Verification items for this drawing (mm, ordinates from the low corner). A direction names the side the tool comes from. Round coordinates to 2 decimals unless told otherwise and drop trailing zeros. Write each loop counter-clockwise with the first axis right and the second up, starting at its lowest first coordinate (ties: lowest second). Pieces come first, ordered by that corner, then holes. Notation, with made-up numbers: (15, 62) -> (30, 62) arc R20 cw to (30, 86) -> close; hole circle Ø6 at (75, -13). An arc over 180 degrees is marked (long way). One line per item, written item: value.
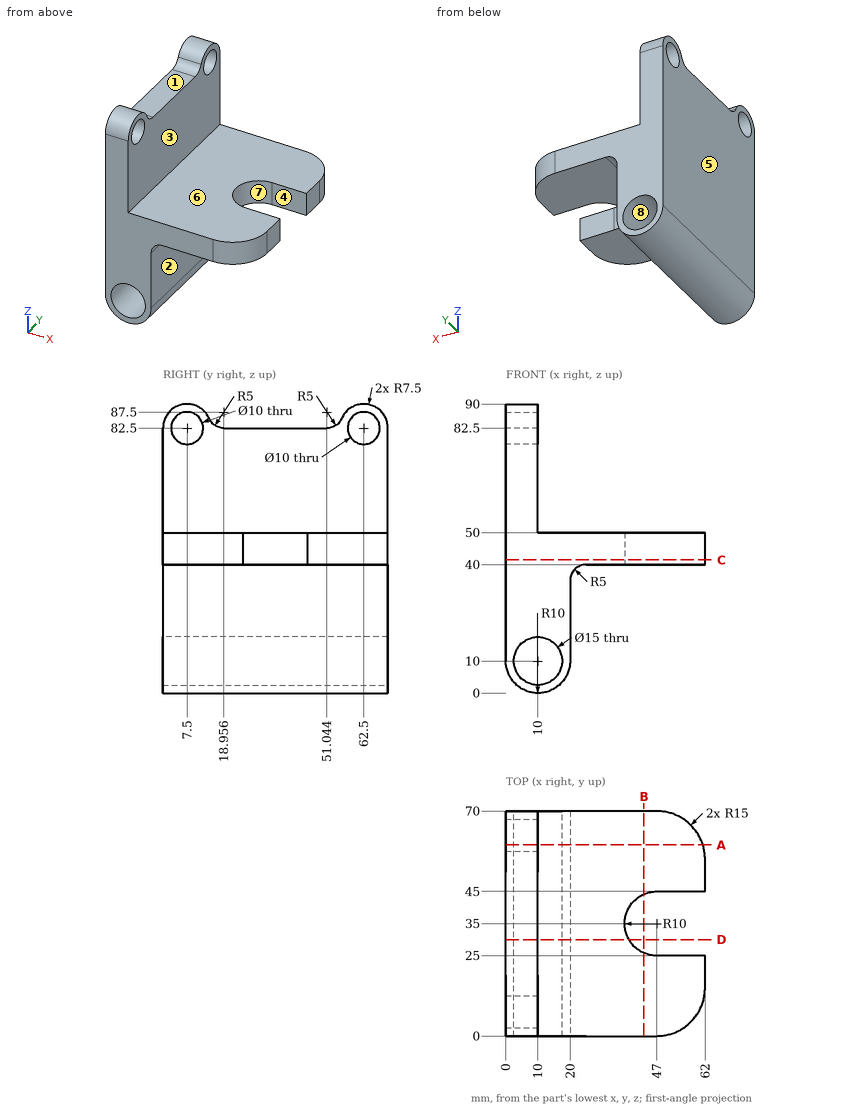
Item 1: Depth check by flat-ended pin: pin 1 (3 mm diameter, centred on x = 13.5, y = 32, fed in from +Z); pin 2 (9 mm diameter, centred on x = 10, z = 10, fed in from +Y); pin 3 (12 mm diameter, centred on x = 28.5, y = 62, fed in from -Z); pin 4 (3 mm diameter, centred on x = 58, z = 45, fed in from +Y). Enter the tip coordinate at first touch or a pass-through.
Result set:
pin 1: z = 50
pin 2: through
pin 3: z = 39.33
pin 4: y = 66.61
Item 2: Sectioned sample at A-A (y = 59.5). Enter the section's corners in (x, z).
Result set:
outline: (0, 10) arc R10 ccw to (20, 10) -> (20, 35) arc R5 cw to (25, 40) -> (61.31, 40) -> (61.31, 50) -> (10, 50) -> (10, 78.5) -> (0, 78.5) -> close; (0, 86.5) -> (10, 86.5) -> (10, 89.37) -> (0, 89.37) -> close; hole circle Ø15 at (10, 10)
Item 3: Sectioned sample at D-D (y = 30). Enter the section's corners in (x, z).
Result set:
outline: (0, 10) arc R10 ccw to (20, 10) -> (20, 35) arc R5 cw to (25, 40) -> (38.34, 40) -> (38.34, 50) -> (10, 50) -> (10, 82.5) -> (0, 82.5) -> close; hole circle Ø15 at (10, 10)
Item 4: Tool access check on the marked faces 1, 2, 3 and 4. Record the directions out of +Z, -Z, +X, -X, +Y, -Y that give a thin tool (end or side, any length) a straight path to the whole face; none if there is none.
Result set:
face 1: +Z, +X, -X
face 2: -Z, +X, +Y, -Y
face 3: +Z, +X, +Y, -Y
face 4: +Z, -Z, +X
Item 5: Material ranges on line 1 along X through (y, z) = (19.5, 62.5); line 2 along Z through (x, y) = (38, 52.5); line 3 along Z through (x, y) = (4, 40.5), recorded low to high.
Result set:
line 1: 0 to 10
line 2: 40 to 50
line 3: 2 to 5.5, 14.5 to 82.5
Item 6: Release check for a two-part mould opening along X. For the marked faces 5, 6, 7 and 8 record: pulls with the +X half, pulls with the -X half, needs draft (parallel to the pull), parting line crosses it, or undercut.
Result set:
face 5: pulls with the -X half
face 6: needs draft
face 7: pulls with the +X half
face 8: undercut
Item 7: Sectioned sample at C-C (z = 41.5). Enter the section's corners in (x, y).
Result set:
outline: (0, 0) -> (47, 0) arc R15 ccw to (62, 15) -> (62, 25) -> (47, 25) arc R10 cw to (47, 45) -> (62, 45) -> (62, 55) arc R15 ccw to (47, 70) -> (0, 70) -> close
Item 8: Sectioned sample at B-B (x = 43). Enter the section's corners in (y, z) (1 decimal).
Result set:
outline: (0, 40) -> (25.8, 40) -> (25.8, 50) -> (0, 50) -> close; (44.2, 40) -> (70, 40) -> (70, 50) -> (44.2, 50) -> close
